from build123d import *

# Parameters (mm, degrees)
SKETCH1_R           = 25
BOSS_EXTRUDE1_DEPTH = 14
SKETCH2_W           = 100
SKETCH2_H           = 16
CUT_EXTRUDE1_DEPTH  = 177.694651872


with BuildPart() as part:
    # Sketch1 → Boss-Extrude1 (new body)
    with BuildSketch(Plane.XY):
        with BuildLine():
            Line((-43.801805937, 33.262618608), (-145, -100))
            Line((-145, -100), (55, -100))
            Line((55, -100), (55, 0))
            ThreePointArc((55, 0), (17.548513804, 52.125326505), (-43.801805937, 33.262618608))
        make_face()
        Circle(SKETCH1_R, mode=Mode.SUBTRACT)
    extrude(amount=BOSS_EXTRUDE1_DEPTH)

    # Sketch2 → Cut-Extrude1 (cut, through all)
    with BuildSketch(Plane.XY.offset(14)):
        with Locations((-95, -92)):
            Rectangle(SKETCH2_W, SKETCH2_H)
    extrude(amount=-CUT_EXTRUDE1_DEPTH, mode=Mode.SUBTRACT)


solid = part.part
Verification items for the finished model (mm, model axes). A direction names the side the tool comes from. Coordinates: 2 decimals unless noted, no trailing zeros. Order: outer loops, then holes, each group sorted by start corner. A loop starts at its lowest first (then second) coordinate and runs counter-clockwise, first axis right, second up.
1. Sectioned sample at D-D, the plane y = -89.5. Record the cut outline in (x, z).
Results found:
outline: (-45, 0) - (55, 0) - (55, 14) - (-45, 14) - close
2. Sectioned sample at A-A, the plane z = 10. Record the cut outline in (x, y), and give its area (3 significant figures).
Results found:
outline: (-132.85, -84) - (-45, -84) - (-45, -100) - (55, -100) - (55, 0) arc R55 ccw to (-43.8, 33.26) - close; hole circle Ø50 at (0, 0)
area: 17,700 mm2
3. Sectioned sample at B-B, the plane x = 0. Record the cut outline in (y, z).
Results found:
outline: (-100, 0) - (-25, 0) - (-25, 14) - (-100, 14) - close; (25, 0) - (55, 0) - (55, 14) - (25, 14) - close
4. Release check for a two-part mould opening along X. For faces 3 (the face through (-90, -84, 7)), 4 (the face through (55, -51, 7)), 5 (the face through (23.846, 7.509, 6.902)) record: +X half, -X half, draft (parallel to the pull), parting line (faces both ways), or undercut.
Results found:
face 3: draft
face 4: +X half
face 5: undercut
5. Sectioned sample at C-C, the plane y = -8. Record the cut outline in (x, z).
Results found:
outline: (-75.14, 0) - (-23.69, 0) - (-23.69, 14) - (-75.14, 14) - close; (23.69, 0) - (55, 0) - (55, 14) - (23.69, 14) - close
6. Go/stop test with flat-tipped pins: pin 1 Ø4 at (y, z) = (-14.5, 11) entering from -X; pin 2 Ø1.5 at (x, z) = (-72.5, 10) entering from -Y; pin 3 Ø8 at (x, z) = (-39, 10) entering from +Y. Record where each tip stops, or that it passes through.
Results found:
pin 1: stops at x = -81.59
pin 2: stops at y = -84
pin 3: stops at y = 42.43
7. Scan lines: line 1 (Y direction, x = 0, z = 4.75); line 2 (X direction, y = -20, z = 6.75); line 3 (Y direction, x = 18, z = 12.5). Record each from-to range of solid material in increasing order.
Results found:
line 1: y = -100 to -25, 25 to 55
line 2: x = -84.25 to -15, 15 to 55
line 3: y = -100 to -17.35, 17.35 to 51.97
8. Set-up check for faces 1 (the face through (18.46, 51.81, 6.9)), 2 (the face through (-45, -92, 7)): record each of +Z, -Z, +X, -X, +Y, -Y from which the full face is reachable in a straight line by a thin tool's end or side.
Results found:
face 1: +Z, -Z, +Y
face 2: +Z, -Z, -X, -Y
